```python
from build123d import *

# Parameters (mm, degrees)
SKETCH2_W          = 12.434421081
SKETCH2_H          = 11.052818739
CUT_EXTRUDE2_DEPTH = 6
CUT_EXTRUDE3_DEPTH = 3
CHAMFER1_SIZE      = 1


with BuildPart() as part:
    # Sketch1 → Revolve1 (revolve)
    with BuildSketch(Plane.XY, mode=Mode.PRIVATE) as revolve1_sk:
        Polygon((0, 0), (3, 0), (3, 16), (5, 16), (5, 22), (0, 22), (0, 0.812520437), align=None)
    revolve(revolve1_sk.sketch.rotate(Axis((0, 22, 0), (0, -1, 0)), 90), axis=Axis((0, 22, 0), (0, -1, 0)))

    # Sketch2 → Cut-Extrude2 (cut)
    with BuildSketch(Plane(origin=(0, 22, 0), x_dir=(1, 0, 0), z_dir=(0, 1, 0))):
        with Locations((0.708980149, -0.054536934)):
            Rectangle(SKETCH2_W, SKETCH2_H)
        Polygon((5, 0), (2.5, 4.330127019), (-2.5, 4.330127019), (-5, 0), (-2.5, -4.330127019), (2.5, -4.330127019), align=None, mode=Mode.SUBTRACT)
    extrude(amount=-CUT_EXTRUDE2_DEPTH, mode=Mode.SUBTRACT)

    # Sketch3 → Cut-Extrude3 (cut)
    with BuildSketch(Plane(origin=(0, 22, 0), x_dir=(1, 0, 0), z_dir=(0, 1, 0))):
        Polygon((3, 0), (1.5, 2.598076211), (-1.5, 2.598076211), (-3, 0), (-1.5, -2.598076211), (1.5, -2.598076211), align=None)
    extrude(amount=-CUT_EXTRUDE3_DEPTH, mode=Mode.SUBTRACT)

    # Sketch5 → Cut-Loft1 section 0
    with BuildSketch(Plane(origin=(0, 19, 0), x_dir=(1, 0, 0), z_dir=(0, 1, 0)), mode=Mode.PRIVATE) as cut_loft1_s0:
        with BuildLine():
            Line((1.5, 2.598076211), (-1.5, 2.598076211))
            Line((-1.5, 2.598076211), (-3, 0))
            Line((-3, 0), (-1.5, -2.598076211))
            Line((-1.5, -2.598076211), (1.5, -2.598076211))
            Line((1.5, -2.598076211), (3, 0))
            Line((3, 0), (1.5, 2.598076211))
        make_face()
    loft([cut_loft1_s0.sketch, Vertex(0, 17.68563071, 0)], mode=Mode.SUBTRACT)

    # Chamfer1
    chamfer1_edges = [part.edges().sort_by_distance(p)[0] for p in [
        (0, 0, -3),
    ]]
    chamfer(chamfer1_edges, length=CHAMFER1_SIZE)

    # Sketch6 → Cut-Revolve1 (revolve, cut)
    with BuildSketch(Plane(origin=(0, 0, 0), x_dir=(0, 0, -1), z_dir=(1, 0, 0)), mode=Mode.PRIVATE) as cut_revolve1_sk:
        with BuildLine():
            Line((-5.464509536, 21.264956491), (-5.887873992, 22.169745092))
            Line((-5.887873992, 22.169745092), (-3.885003272, 23.64244415))
            Line((-3.885003272, 23.64244415), (-2.598076211, 22))
            ThreePointArc((-2.598076211, 22), (-4.060125505, 21.744916236), (-5.464509536, 21.264956491))
        make_face()
    revolve(cut_revolve1_sk.sketch.rotate(Axis((0, 16, 0), (0, 1, 0)), 149.999999986), axis=Axis((0, 16, 0), (0, 1, 0)), mode=Mode.SUBTRACT)


solid = part.part
```
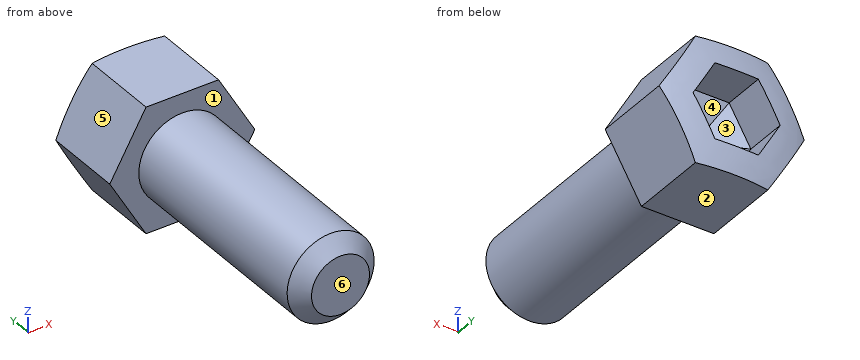
Geometry check sheet. Reference: the model listing, model coordinates, mm. Face numbers are marked on the shaded views. A direction names the side the tool comes from. Give positions to 0.01 mm unless a question says otherwise; leave off trailing zeros. Loops run counter-clockwise (first coordinate to the right, second up) from the corner with the lowest first, then second, coordinate; pieces in that order, holes last. Notation, with made-up numbers: M 20.5,-14.5 L 57.5,-14.5 A16 cw 57.5,13.5 Z; hole C -31.75,-28.75 d3. An arc over 180 degrees is marked long. Write item = value, one per line. Start each with the question number.
1. Section check A-A, the plane y = 17.25. Enter the section's corners in (x, z), plus the area to 3 significant figures.
2. Thickness scan on probe 1 along X at (y, z) = (18.75, 0.25); probe 2 along X at (y, z) = (19.5, -2.5); probe 3 along Y at (x, z) = (-0.5, -1). Record the ranges inside material, lowest first.
3. Go/stop test with flat-tipped pins: P1, Ø1.5, axis at x = 3.5, z = -0.5, coming from the -Y side; P2, Ø3, axis at x = -0.5, z = 2.5, coming from the +Y side; P3, Ø5, axis at x = -3.5, y = 9.5, coming from the -Z side; P4, Ø4, axis at y = 8, z = -3, coming from the +X side. Record where each tip stops, or that it passes through.
4. Tool access check on the marked faces 1, 2 and 3. Record the directions out of +Z, -Z, +X, -X, +Y, -Y that give a thin tool (end or side, any length) a straight path to the whole face; none if there is none.
5. Draft check along X on the marked faces 4, 5 and 6. Enter one of: +X half, -X half, draft (parallel to the pull), parting line (faces both ways), or undercut.
6. Section check B-B, the plane y = 7. Enter the section's corners in (x, z).
Values follow:
q1.outline = M -5,0 L -2.5,-4.33 L 2.5,-4.33 L 5,0 L 2.5,4.33 L -2.5,4.33 Z
q1.area = 65.0 mm^2
q2.probe_1 = -4.86 to -2.29, 2.29 to 4.86
q2.probe_2 = -3.56 to -1.56, 1.56 to 3.56
q2.probe_3 = 0 to 18.19
q3.P1 = 0.79
q3.P2 = 22
q3.P3 = -2.83
q3.P4 = 2.83
q4.face_1 = -Y
q4.face_2 = -Z, +X, -X, +Y, -Y
q4.face_3 = +Y
q5.face_4 = undercut
q5.face_5 = -X half
q5.face_6 = draft
q6.outline = C 0,0 d6
